from build123d import *

# Parameters (mm, degrees)
ROUND_FLANGE_SKETCH_R            = 50
ROUND_FLANGE_100_DEPTH           = 15
ROUND_FLANGE_BOLT_HOLES_SKETCH_R = 5
ROUND_FLANGE_BOLT_HOLES_DEPTH    = 15
SPOOL_CORE_SKETCH_R              = 18
SPOOL_CORE_36_DEPTH              = 85
CORE_START                       = -85
CORE_BORE_SKETCH_R               = 18
CORE_BORE_36_DEPTH               = 85
SPOOL_PIPE_SKETCH_R              = 25
SPOOL_PIPE_50_DEPTH              = 85
OVAL_FLANGE_DEPTH                = 15
OVAL_FLANGE_HOLES_SKETCH_R       = 6.5
OVAL_FLANGE_HOLES_2X_13_DEPTH    = 15
OVAL_FLANGE_BORE_SKETCH_R        = 18
OVAL_FLANGE_BORE_36_DEPTH        = 40
THROUGH_BORE_SKETCH_R            = 14
THROUGH_BORE_28_DEPTH            = 75


with BuildPart() as part:
    # Round Flange Sketch → Round Flange Ø100 (new body)
    with BuildSketch(Plane.XY):
        Circle(ROUND_FLANGE_SKETCH_R)
    extrude(amount=ROUND_FLANGE_100_DEPTH)

    # Round Flange Bolt Holes Sketch → Round Flange Bolt Holes (cut)
    with BuildSketch(Plane.XY.offset(15)):
        with Locations((-30.310889132, 17.5)):
            Circle(ROUND_FLANGE_BOLT_HOLES_SKETCH_R)
        with Locations((0, 35)):
            Circle(ROUND_FLANGE_BOLT_HOLES_SKETCH_R)
        with Locations((30.310889132, 17.5)):
            Circle(ROUND_FLANGE_BOLT_HOLES_SKETCH_R)
        with Locations((-30.310889132, -17.5)):
            Circle(ROUND_FLANGE_BOLT_HOLES_SKETCH_R)
        with Locations((30.310889132, -17.5)):
            Circle(ROUND_FLANGE_BOLT_HOLES_SKETCH_R)
        with Locations((0, -35)):
            Circle(ROUND_FLANGE_BOLT_HOLES_SKETCH_R)
    extrude(amount=-ROUND_FLANGE_BOLT_HOLES_DEPTH, mode=Mode.SUBTRACT)

    # Spool Core Sketch → Spool Core Ø36 (add)
    with BuildSketch(Plane.XY.offset(15)):
        Circle(SPOOL_CORE_SKETCH_R)
    extrude(amount=SPOOL_CORE_36_DEPTH)

    # Core Bore Sketch → Core Bore Ø36 (cut)
    with BuildSketch(Plane.XY.offset(100).offset(CORE_START)):
        Circle(CORE_BORE_SKETCH_R)
    extrude(amount=CORE_BORE_36_DEPTH, mode=Mode.SUBTRACT)

    # Spool Pipe Sketch → Spool Pipe Ø50 (add)
    with BuildSketch(Plane.XY.offset(15)):
        Circle(SPOOL_PIPE_SKETCH_R)
    extrude(amount=SPOOL_PIPE_50_DEPTH)

    # Oval Flange Sketch → Oval Flange (add)
    with BuildSketch(Plane.XY.offset(100)):
        with BuildLine():
            Line((-28.618176043, 9), (-14.309088021, 54.5))
            ThreePointArc((-14.309088021, 54.5), (0, 65), (14.309088021, 54.5))
            Line((14.309088021, 54.5), (28.618176043, 9))
            ThreePointArc((28.618176043, 9), (30, 0), (28.618176043, -9))
            Line((28.618176043, -9), (14.309088021, -54.5))
            ThreePointArc((14.309088021, -54.5), (0, -65), (-14.309088021, -54.5))
            Line((-14.309088021, -54.5), (-28.618176043, -9))
            ThreePointArc((-28.618176043, -9), (-30, 0), (-28.618176043, 9))
        make_face()
    extrude(amount=OVAL_FLANGE_DEPTH)

    # Oval Flange Holes Sketch → Oval Flange Holes 2xØ13 (cut)
    with BuildSketch(Plane.XY.offset(115)):
        with Locations((0, 50)):
            Circle(OVAL_FLANGE_HOLES_SKETCH_R)
        with Locations((0, -50)):
            Circle(OVAL_FLANGE_HOLES_SKETCH_R)
    extrude(amount=-OVAL_FLANGE_HOLES_2X_13_DEPTH, mode=Mode.SUBTRACT)

    # Oval Flange Bore Sketch → Oval Flange Bore Ø36 (cut)
    with BuildSketch(Plane.XY.offset(115)):
        Circle(OVAL_FLANGE_BORE_SKETCH_R)
    extrude(amount=-OVAL_FLANGE_BORE_36_DEPTH, mode=Mode.SUBTRACT)

    # Through Bore Sketch → Through Bore Ø28 (cut)
    with BuildSketch(Plane.XY.offset(75)):
        Circle(THROUGH_BORE_SKETCH_R)
    extrude(amount=-THROUGH_BORE_28_DEPTH, mode=Mode.SUBTRACT)


solid = part.part
Input: part model. Units: mm. Frame: model coordinates. A direction names the side the tool comes from. Coordinates: 2 decimals unless noted, no trailing zeros. Loops run counter-clockwise (first coordinate to the right, second up) from the corner with the lowest first, then second, coordinate; pieces in that order, holes last.
Q1. Cut plane C-C (x = 0). Give the number of separate pieces and of enclosed holes in the cut face, then the cut area to 3 significant figures.
Q2. Cut plane B-B (z = 60). Output: boundary loops of the cut face in (x, y), then the cut area to 3 significant figures.
Q3. Cut plane D-D (y = 20.5). Output: boundary loops of the cut face in (x, z).
Q4. Cut plane A-A (y = 0). Output: boundary loops of the cut face in (x, z).
Q5. Set-up query: faces 1 (the face through (21.564, -31.432, 107.395)), 2 (the face through (-1.409, -56.345, 107.605)), 3 (the face through (-22.9, -10.4, 15)), 4 (the face through (47.69, 15.02, 7.4)), 5 (the face through (-30, 0, 107)). Return all of +Z, -Z, +X, -X, +Y, -Y with unobstructed straight access to the full face (end or side cutting, diameter ignored); none if empty.
Q6. Contact query for flat-ended pins moving along their axis: pin 1 (16 mm diameter, centred on x = 30.31, y = -17.5, fed in from +Z); pin 2 (8 mm diameter, centred on y = -16.5, z = 17, fed in from +X); pin 3 (3 mm diameter, centred on y = 15.5, z = 75, fed in from -X); pin 4 (5 mm diameter, centred on y = -1, z = 40, fed in from -X). Output: stop coordinate, or through.
Q7. Draft query along Y for faces 6 (the face through (21.363, 32.068, 107.395)), 7 (the face through (3, 39, 8)), 8 (the face through (30, 0, 107)). Return one class per face: +Y half, -Y half, draft (parallel to the pull), parting line (faces both ways), or undercut.
Q8. Material intervals for line 1 (Y direction, x = 0, z = 8.5); line 2 (Z direction, x = -23.5, y = -21.5); line 3 (Y direction, x = 0, z = 106), sorted ascending.
Working result:
1. separate pieces: 6
1. enclosed holes: 0
1. area: 3,470 mm2
2. outline: circle Ø50 at (0, 0); hole circle Ø28 at (0, 0)
2. area: 1,350 mm2
3. outline: (-45.6, 0) - (-34.31, 0) - (-34.31, 15) - (-45.6, 15) - close; (-26.31, 0) - (26.31, 0) - (26.31, 15) - (14.31, 15) - (14.31, 100) - (25, 100) - (25, 115) - (-25, 115) - (-25, 100) - (-14.31, 100) - (-14.31, 15) - (-26.31, 15) - close; (34.31, 0) - (45.6, 0) - (45.6, 15) - (34.31, 15) - close
4. outline: (-50, 0) - (-14, 0) - (-14, 75) - (-18, 75) - (-18, 115) - (-30, 115) - (-30, 100) - (-25, 100) - (-25, 15) - (-50, 15) - close; (14, 0) - (50, 0) - (50, 15) - (25, 15) - (25, 100) - (30, 100) - (30, 115) - (18, 115) - (18, 75) - (14, 75) - close
5. face 1: +Z, +X, -Y
5. face 2: +Z
5. face 3: none
5. face 4: -Z
5. face 5: +Z, -X
6. pin 1: stops at z = 115
6. pin 2: stops at x = 48.27
6. pin 3: stops at x = -20.71
6. pin 4: stops at x = -25
7. face 6: +Y half
7. face 7: undercut
7. face 8: parting line
8. line 1: y = -50 to -40, -30 to -14, 14 to 30, 40 to 50
8. line 2: z = 0 to 15, 100 to 115
8. line 3: y = -65 to -56.5, -43.5 to -18, 18 to 43.5, 56.5 to 65
